```python
from build123d import *

# Parameters (mm, degrees)
G1_TAPPED_HOLE1_D = 30.75
CHAMFER1_SIZE     = 1


with BuildPart() as part:
    # Sketch1 → Revolve1 (revolve)
    with BuildSketch(Plane(origin=(0, 0, 0), x_dir=(0, 0, -1), z_dir=(1, 0, 0)), mode=Mode.PRIVATE) as revolve1_sk:
        Polygon((0, 0), (0, 20), (-10, 20), (-10, 25), (-20, 25), (-20, 0), align=None)
    revolve(revolve1_sk.sketch.rotate(Axis((0, 0, 20), (0, 0, -1)), 90), axis=Axis((0, 0, 20), (0, 0, -1)))

    # G1 Tapped Hole1 (through all)
    with Locations(Plane.XY.offset(20)):
        with Locations((0, 0)):
            Hole(G1_TAPPED_HOLE1_D / 2)

    # Chamfer1
    chamfer1_edges = [part.edges().sort_by_distance(p)[0] for p in [
        (-25, 0, 20),
    ]]
    chamfer(chamfer1_edges, length=CHAMFER1_SIZE)


solid = part.part
```
Here's how the part is built. I have some questions about the finished solid (model axes, mm). A direction names the side the tool comes from. Give positions to 0.01 mm unless a question says otherwise; leave off trailing zeros. Loops run counter-clockwise (first coordinate to the right, second up) from the corner with the lowest first, then second, coordinate; pieces in that order, holes last. Notation, with made-up numbers: (59, 35.25) -> (66, 35.25) arc R21 cw to (66, 45.25) -> close; hole circle Ø3 at (57.5, 24.5). An arc over 180 degrees is marked (long way). Use one line per item in the form item = value. Start each with the question number.
1) Imagine slicing it at C-C (z = 17.5). Please give me the cut outline in (x, y) (3 decimals).
2) Please list where these lines run through material, in increasing order: line 1 along Y through (x, z) = (0, 6.5) (3 decimals); line 2 along Y through (x, z) = (0, 10.25) (3 decimals); line 3 along X through (y, z) = (11, 2.5).
3) Imagine slicing it at A-A (x = 0). Please give me the cut outline in (y, z) (3 decimals), then the cut area to 3 significant figures.
4) For P1, Ø2, axis at y = 8.5, z = 6, coming from the +X side; P2, Ø12, axis at x = 14.5, z = 15, coming from the -Y side; P3, Ø6, axis at x = 4.5, z = 15, coming from the +Y side, each with a flat end and sliding along its axis, tell me the tip position at first contact or that it passes through.
5) Which directions (+Z, -Z, +X, -X, +Y, -Y) give clear straight access to the entire face, cutting with the end or side of a thin tool? Please do faces 1 (the face through (11, -17, 10)), 2 (the face through (23.846, -7.509, 14.563)).
6) Imagine slicing it at D-D (z = 8.5). Please give me the cut outline in (x, y) (3 decimals), then the cut area to 3 significant figures.
Check values:
q1.outline = circle Ø50 at (0, 0); hole circle Ø30.75 at (0, 0)
q2.line_1 = -20 to -15.375, 15.375 to 20
q2.line_2 = -25 to -15.375, 15.375 to 25
q2.line_3 = -16.7 to -10.74, 10.74 to 16.7
q3.outline = (-25, 10) -> (-20, 10) -> (-20, 0) -> (-15.375, 0) -> (-15.375, 20) -> (-24, 20) -> (-25, 19) -> close; (15.375, 0) -> (20, 0) -> (20, 10) -> (25, 10) -> (25, 19) -> (24, 20) -> (15.375, 20) -> close
q3.area = 284 mm^2
q4.P1 = 18.54
q4.P2 = -23.51
q4.P3 = 24.95
q5.face_1 = -Z
q5.face_2 = +Z, -Z
q6.outline = circle Ø40 at (0, 0); hole circle Ø30.75 at (0, 0)
q6.area = 514 mm^2
